Source: CAD feature listing. Evaluate the final solid. Frame: model axes, mm. A direction names the side the tool comes from. Give positions to 0.01 mm unless a question says otherwise; leave off trailing zeros. Loops run counter-clockwise (first coordinate to the right, second up) from the corner with the lowest first, then second, coordinate; pieces in that order, holes last. Notation, with made-up numbers: M 39.25,-35.5 L 45.25,-35.5 A28 cw 45.25,-13.5 Z; hole C -2.75,35 d6. An arc over 180 degrees is marked long. Put each result on its own line as item: value.
from build123d import *

# Parameters (mm, degrees)
SKETCH1_W                                           = 80
SKETCH1_H                                           = 150
BOSS_EXTRUDE1_DEPTH                                 = 14
HOLE_SIZE_BY_SOCKET_HEAD_CAP_SCREW_TYPE_D           = 11
HOLE_SIZE_BY_SOCKET_HEAD_CAP_SCREW_TYPE_CBORE_D     = 18
HOLE_SIZE_BY_SOCKET_HEAD_CAP_SCREW_TYPE_CBORE_DEPTH = 8
CHAMFER1_SIZE                                       = 5


with BuildPart() as part:
    # Sketch1 → Boss-Extrude1 (new body)
    with BuildSketch(Plane(origin=(0, 0, 0), x_dir=(1, 0, 0), z_dir=(0, 1, 0))):
        with Locations((40, 75)):
            Rectangle(SKETCH1_W, SKETCH1_H)
    extrude(amount=BOSS_EXTRUDE1_DEPTH)

    # Hole size (by socket head cap screw type)1 (through all)
    with Locations(Plane(origin=(0, 14, 0), x_dir=(1, 0, 0), z_dir=(0, 1, 0))):
        with Locations((25, 130), (25, 20)):
            CounterBoreHole(HOLE_SIZE_BY_SOCKET_HEAD_CAP_SCREW_TYPE_D / 2, HOLE_SIZE_BY_SOCKET_HEAD_CAP_SCREW_TYPE_CBORE_D / 2, HOLE_SIZE_BY_SOCKET_HEAD_CAP_SCREW_TYPE_CBORE_DEPTH)

    # Chamfer1
    chamfer1_edges = [part.edges().sort_by_distance(p)[0] for p in [
        (0, 7, -150),
        (0, 7, 0),
    ]]
    chamfer(chamfer1_edges, length=CHAMFER1_SIZE)


solid = part.part
1. Section query B-B (y = 3). Output: boundary loops of the cut face in (x, z), plus the area to 3 significant figures.
Found:
outline: M 0,-145 L 5,-150 L 80,-150 L 80,0 L 5,0 L 0,-5 Z; hole C 25,-130 d11; hole C 25,-20 d11
area: 11,800 mm^2
2. Access query for faces 1 (the cylindrical face through (33.584, 10.056, -22.703)), 2 (the flat face through (42, 7, -150)). Directions: +Z, -Z, +X, -X, +Y, -Y. A direction counts if a zero-diameter tool reaches every point of the face in a straight line with its end or side. Return the directions, or none.
Found:
face 1: +Y
face 2: -Z, +X, -X, +Y, -Y
3. Material intervals for line 1 (Z direction, x = 25, y = 9.75); line 2 (Z direction, x = 25, y = 2.7); line 3 (X direction, y = 10.75, z = -130), sorted ascending. Write a range as from..to.
Found:
line 1: -150..-139, -121..-29, -11..0
line 2: -150..-135.5, -124.5..-25.5, -14.5..0
line 3: 0..16, 34..80
4. Draft query along Z for faces 3 (the flat face through (3, 7, -2)), 4 (the flat face through (39, 0, -76)), 5 (the cylindrical face through (22.043, 2.958, -24.638)). Return one class per face: pulls with the +Z half, pulls with the -Z half, needs draft (parallel to the pull), parting line crosses it, or undercut.
Found:
face 3: pulls with the +Z half
face 4: needs draft
face 5: undercut
5. Contact query for flat-ended pins moving along their axis: P1, Ø14.5, axis at x = 25.5, z = -20, coming from the +Y side; P2, Ø6.5, axis at x = 25, z = -130, coming from the -Y side. Output: stop coordinate, or through.
Found:
P1: y = 6
P2: through
6. Section query A-A (z = -130). Output: boundary loops of the cut face in (x, y).
Found:
outline: M 0,0 L 19.5,0 L 19.5,6 L 16,6 L 16,14 L 0,14 Z; M 30.5,0 L 80,0 L 80,14 L 34,14 L 34,6 L 30.5,6 Z
7. Section query C-C (x = 25). Output: boundary loops of the cut face in (y, z).
Found:
outline: M 0,-150 L 14,-150 L 14,-139 L 6,-139 L 6,-135.5 L 0,-135.5 Z; M 0,-124.5 L 6,-124.5 L 6,-121 L 14,-121 L 14,-29 L 6,-29 L 6,-25.5 L 0,-25.5 Z; M 0,-14.5 L 6,-14.5 L 6,-11 L 14,-11 L 14,0 L 0,0 Z
